```python
from build123d import *

# Parameters (mm, degrees)
SKETCH1_W           = 200
SKETCH1_H           = 200
SKETCH1_R           = 2
BOSS_EXTRUDE1_DEPTH = 8
SKETCH2_R           = 2.5
CUT_EXTRUDE1_DEPTH  = 283.955826941
CUT_EXTRUDE2_DEPTH  = 283.955826941


with BuildPart() as part:
    # Sketch1 → Boss-Extrude1 (new body)
    with BuildSketch(Plane(origin=(0, 0, 0), x_dir=(1, 0, 0), z_dir=(0, 1, 0))):
        with Locations((100, 100)):
            Rectangle(SKETCH1_W, SKETCH1_H)
        with Locations(Location((195, 195, 0), (0, 0, 270))):
            Circle(SKETCH1_R, mode=Mode.SUBTRACT)
        with Locations(Location((5, 195, 0), (0, 0, 270))):
            Circle(SKETCH1_R, mode=Mode.SUBTRACT)
        with Locations(Location((5, 5, 0), (0, 0, 270))):
            Circle(SKETCH1_R, mode=Mode.SUBTRACT)
        with Locations(Location((195, 5, 0), (0, 0, 270))):
            Circle(SKETCH1_R, mode=Mode.SUBTRACT)
    extrude(amount=BOSS_EXTRUDE1_DEPTH)

    # Sketch2 → Cut-Extrude1 (cut, through all)
    with BuildSketch(Plane.XZ):
        with Locations(Location((187.5, -49.5, 0), (0, 0, 270))):
            Circle(SKETCH2_R)
        with Locations(Location((157.5, -49.5, 0), (0, 0, 270))):
            Circle(SKETCH2_R)
        with Locations(Location((80, -120, 0), (0, 0, 270))):
            Circle(SKETCH2_R)
        with Locations(Location((80, -80, 0), (0, 0, 270))):
            Circle(SKETCH2_R)
        with Locations(Location((120, -80, 0), (0, 0, 270))):
            Circle(SKETCH2_R)
        with Locations(Location((120, -120, 0), (0, 0, 270))):
            Circle(SKETCH2_R)
        with Locations(Location((42.5, -100, 0), (0, 0, 270))):
            Circle(SKETCH2_R)
        with Locations(Location((12.5, -100, 0), (0, 0, 270))):
            Circle(SKETCH2_R)
        with Locations(Location((157.5, -150.5, 0), (0, 0, 270))):
            Circle(SKETCH2_R)
        with Locations(Location((187.5, -150.5, 0), (0, 0, 270))):
            Circle(SKETCH2_R)
    extrude(amount=-CUT_EXTRUDE1_DEPTH, mode=Mode.SUBTRACT)

    # Sketch3 → Cut-Extrude2 (cut, through all)
    with BuildSketch(Plane(origin=(0, 8, 0), x_dir=(1, 0, 0), z_dir=(0, 1, 0))):
        Polygon((42.5, 200), (75, 160), (125, 160), (157.5, 200), align=None)
        Polygon((42.5, 0), (157.5, 0), (125, 40), (75, 40), align=None)
        with BuildLine():
            Line((19, 85), (19, 115))
            ThreePointArc((19, 115), (27.5, 123.5), (36, 115))
            Line((36, 115), (36, 85))
            ThreePointArc((36, 85), (27.5, 76.5), (19, 85))
        make_face()
        with BuildLine():
            Line((181, 34.5), (181, 64.5))
            ThreePointArc((181, 64.5), (172.5, 73), (164, 64.5))
            Line((164, 64.5), (164, 34.5))
            ThreePointArc((164, 34.5), (172.5, 26), (181, 34.5))
        make_face()
        with BuildLine():
            Line((181, 165.5), (181, 135.5))
            ThreePointArc((181, 135.5), (172.5, 127), (164, 135.5))
            Line((164, 135.5), (164, 165.5))
            ThreePointArc((164, 165.5), (172.5, 174), (181, 165.5))
        make_face()
    extrude(amount=-CUT_EXTRUDE2_DEPTH, mode=Mode.SUBTRACT)


solid = part.part
```
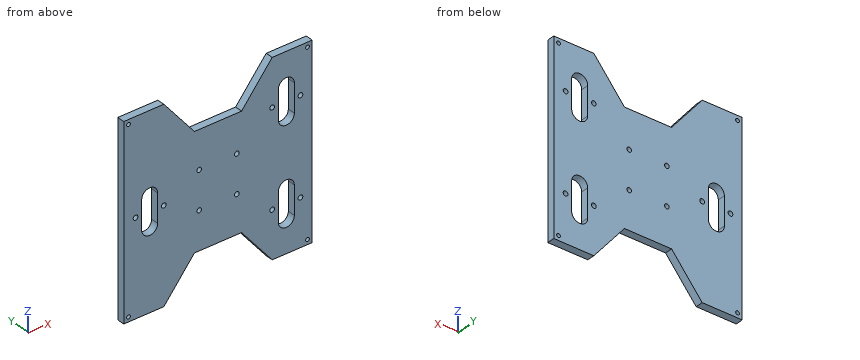
Geometry check sheet. Reference: the model listing, model coordinates, mm. Give positions to 0.01 mm unless a question says otherwise; leave off trailing zeros. Order: outer loops, then holes, each group sorted by start corner. A loop starts at its lowest first (then second) coordinate and runs counter-clockwise, first axis right, second up.
1. Section check B-B, the plane x = 12.5. Enter the section's corners in (y, z).
2. Section check C-C, the plane x = 104.5. Enter the section's corners in (y, z).
3. Thickness scan on L1, parallel to X at y = 6.25, z = -150.5; L2, parallel to Z at x = 157.5, y = 6.5; L3, parallel to Z at x = 195, y = 2.75. Record the ranges inside material, lowest first.
4. Gauge pin test, flat ends, axial feed: pin 1 Ø6 at (x, z) = (164.5, -162) entering from -Y; pin 2 Ø4 at (x, y) = (77.5, 6.5) entering from -Z. Record the tip position at first contact, or that the pin passes through.
5. Section check A-A, the plane z = -89.5. Enter the section's corners in (x, y).
6. Section check D-D, the plane y = 4.25. Give the number of separate pieces and of enclosed holes in the cut face, and give its area (3 significant figures).
Values follow:
1. outline: (0, -200) - (8, -200) - (8, -102.5) - (0, -102.5) - close; (0, -97.5) - (8, -97.5) - (8, 0) - (0, 0) - close
2. outline: (0, -160) - (8, -160) - (8, -40) - (0, -40) - close
3. L1: x = 0 to 155, 160 to 164, 181 to 185, 190 to 200
3. L2: z = -200 to -153, -148 to -52, -47 to 0
3. L3: z = -200 to -197, -193 to -7, -3 to 0
4. pin 1: stops at y = 0
4. pin 2: stops at z = -160
5. outline: (0, 0) - (19, 0) - (19, 8) - (0, 8) - close; (36, 0) - (200, 0) - (200, 8) - (36, 8) - close
6. separate pieces: 1
6. enclosed holes: 17
6. area: 30,900 mm2
